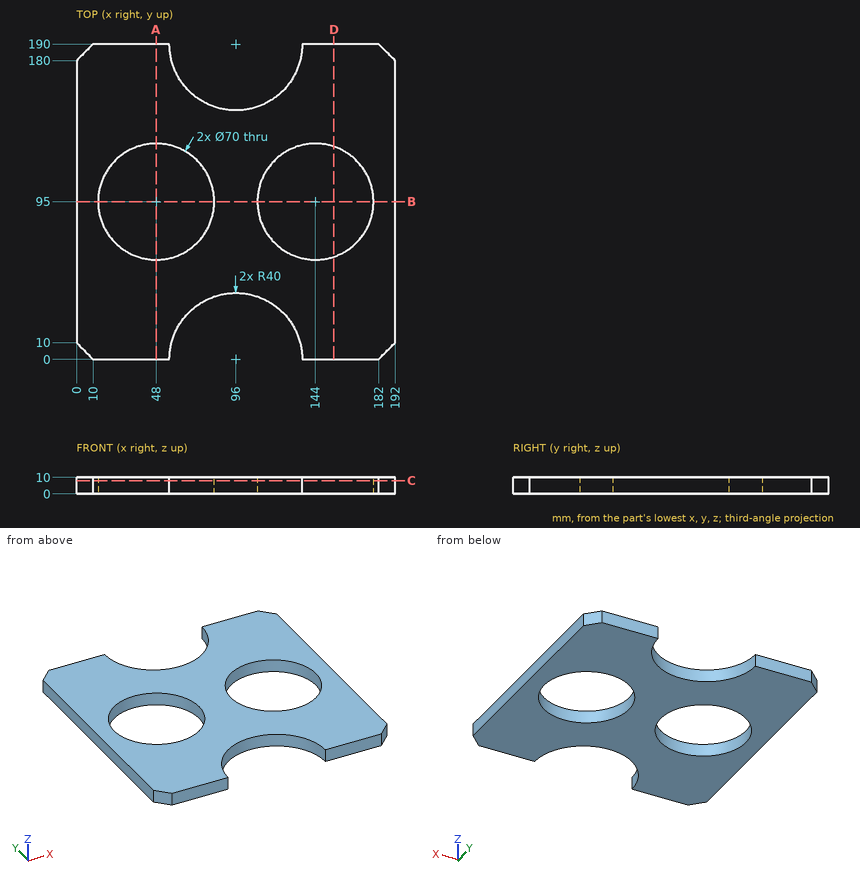
For this review, use the dimensioned drawing (mm, ordinates from the lowest corner) and the shaded views. Give positions to 0.01 mm unless a question says otherwise; leave off trailing zeros. Order: outer loops, then holes, each group sorted by start corner. A loop starts at its lowest first (then second) coordinate and runs counter-clockwise, first axis right, second up.
1) Take a section at B-B (y = 95). Give the boundary of the cut face in (x, z).
2) Take a section at C-C (z = 8). Give the boundary of the cut face in (x, y).
3) Wall thickness on line 1 (X direction, y = 127.5, z = 6.75); line 2 (Y direction, x = 39.5, z = 5.5); line 3 (X direction, y = 164, z = 2.5): over which ranges is each line inside the solid? List them lowest first.
4) Take a section at A-A (x = 48). Give the boundary of the cut face in (y, z), then the cut area to 3 significant figures.
5) Take a section at D-D (x = 155). Give the boundary of the cut face in (y, z).
Derived:
1. outline: (0, 0) - (13, 0) - (13, 10) - (0, 10) - close; (83, 0) - (109, 0) - (109, 10) - (83, 10) - close; (179, 0) - (192, 0) - (192, 10) - (179, 10) - close
2. outline: (0, 10) - (10, 0) - (56, 0) arc R40 cw to (136, 0) - (182, 0) - (192, 10) - (192, 180) - (182, 190) - (136, 190) arc R40 cw to (56, 190) - (10, 190) - (0, 180) - close; hole circle Ø70 at (48, 95); hole circle Ø70 at (144, 95)
3. line 1: x = 0 to 35.01, 60.99 to 131.01, 156.99 to 192
3. line 2: y = 0 to 61.05, 128.95 to 190
3. line 3: x = 0 to 65.6, 126.4 to 192
4. outline: (0, 0) - (60, 0) - (60, 10) - (0, 10) - close; (130, 0) - (190, 0) - (190, 10) - (130, 10) - close
4. area: 1,200 mm2
5. outline: (0, 0) - (61.77, 0) - (61.77, 10) - (0, 10) - close; (128.23, 0) - (190, 0) - (190, 10) - (128.23, 10) - close
